```python
from build123d import *

# Parameters (mm, degrees)
SKETCH1_R           = 200
SKETCH1_R_2         = 20
BOSS_EXTRUDE1_DEPTH = 15
CUT_EXTRUDE1_DEPTH  = 30
FILLET1_R           = 50
SKETCH3_R           = 6.5
CUT_EXTRUDE2_DEPTH  = 50


with BuildPart() as part:
    # Sketch1 → Boss-Extrude1 (new body)
    with BuildSketch(Plane.XY):
        Circle(SKETCH1_R)
        with Locations((0, 156)):
            Circle(SKETCH1_R_2, mode=Mode.SUBTRACT)
        with Locations((135.09996299, -78)):
            Circle(SKETCH1_R_2, mode=Mode.SUBTRACT)
        with Locations((-135.09996299, -78)):
            Circle(SKETCH1_R_2, mode=Mode.SUBTRACT)
    extrude(amount=BOSS_EXTRUDE1_DEPTH)

    # Sketch2 → Cut-Extrude1 (cut)
    with BuildSketch(Plane.XY.offset(15)):
        with BuildLine():
            Line((-45.962666587, -116.432743419), (-177.651298468, -273.373143566))
            Line((-177.651298468, -273.373143566), (100.686015144, -181.64949066))
            Line((100.686015144, -181.64949066), (45.962666587, -116.432743419))
            ThreePointArc((45.962666587, -116.432743419), (0, -95), (-45.962666587, -116.432743419))
        make_face()
        with BuildLine():
            Line((-77.852380339, 98.0212086), (-147.922437807, 290.537109271))
            Line((-147.922437807, 290.537109271), (-207.656081069, 3.62809841))
            Line((-207.656081069, 3.62809841), (-123.815046927, 18.411534819))
            ThreePointArc((-123.815046927, 18.411534819), (-82.27241336, 47.5), (-77.852380339, 98.0212086))
        make_face()
        with BuildLine():
            Line((123.815046927, 18.411534819), (325.573736275, -17.163965705))
            Line((325.573736275, -17.163965705), (106.970065924, 178.021392251))
            Line((106.970065924, 178.021392251), (77.852380339, 98.0212086))
            ThreePointArc((77.852380339, 98.0212086), (82.27241336, 47.5), (123.815046927, 18.411534819))
        make_face()
    extrude(amount=-CUT_EXTRUDE1_DEPTH, mode=Mode.SUBTRACT)

    # Fillet1
    fillet1_edges = [part.edges().sort_by_distance(p)[0] for p in [
        (199.937763867, 4.989045978, 7.5),
        (104.289522491, 170.656659696, 7.5),
        (-104.289522491, 170.656659696, 7.5),
        (-199.937763867, 4.989045978, 7.5),
        (-95.648241376, -175.645705674, 7.5),
        (95.648241376, -175.645705674, 7.5),
    ]]
    fillet(fillet1_edges, radius=FILLET1_R)

    # Sketch3 → Cut-Extrude2 (cut)
    with BuildSketch(Plane.XY.offset(15)):
        with Locations((0, 30)):
            Circle(SKETCH3_R)
        with Locations((25.980762114, -15)):
            Circle(SKETCH3_R)
        with Locations((-25.980762114, -15)):
            Circle(SKETCH3_R)
    extrude(amount=-CUT_EXTRUDE2_DEPTH, mode=Mode.SUBTRACT)


solid = part.part
```
Read the model definition and answer for the solid it produces. Units are mm, in the model's axes. A direction names the side the tool comes from. Coordinates: 2 decimals unless noted, no trailing zeros. Write each loop counter-clockwise with the first axis right and the second up, starting at its lowest first coordinate (ties: lowest second). Pieces come first, ordered by that corner, then holes. Notation, with made-up numbers: (17, -14) - (64, -14) arc R12 ccw to (64, 9) - close; hole circle Ø10 at (-24.75, -38.75). An arc over 180 degrees is marked (long way). Answer as a JSON object with one key per item and string values. Group by question number.
1. A cutting plane is placed at C-C (y = -78). Determine the outline of the cut face in (x, z), plus the area to 3 significant figures.
2. A cutting plane is placed at B-B (z = 11.5). Determine the outline of the cut face in (x, y).
3. Which of the six approach directions +Z, -Z, +X, -X, +Y, -Y give full straight-line access (tool end or side, diameter ignored) to faces 1 (the flat face through (-55.756, -128.104, 7.605)), 2 (the flat face through (-83.063, 112.338, 7.605)), 3 (the flat face through (-3, -16, 0)), 4 (the cylindrical face through (0.8, 200, 7.4)), 5 (the flat face through (83.21, 112.74, 7.6))?
4. A cutting plane is placed at D-D (y = 156). Determine the outline of the cut face in (x, z), plus the area to 3 significant figures.
5. Each of these flat-tipped pins is pushed along its axis until it touches: P1, Ø8, axis at x = 25.98, y = -15, coming from the -Z side; P2, Ø5, axis at x = 133.5, z = 5, coming from the +Y side; P3, Ø4, axis at x = -33.5, z = 11.5, coming from the -Y side; P4, Ø2, axis at y = -39, z = 6.5, coming from the -X side. Where does it stop, or does it pass through?
6. The mould has two halves that part along X. Classify faces 6 (the flat face through (-139.2, 15.7, 7.6)), 7 (the flat face through (56.034, -128.436, 7.605)), 8 (the flat face through (138.819, 15.766, 7.605)): +X half, -X half, draft (parallel to the pull), parting line (faces both ways), or undercut.
7. Consider L1, parallel to Y at x = 0, z = 3.5; L2, parallel to Y at x = -5, z = 6.5; L3, parallel to Y at x = 123.5, z = 5.5. Determine where each line is inside the solid, lowest interval first. Write a range as [from, to].
8. A cutting plane is placed at A-A (x = 0). Determine the outline of the cut face in (y, z).
Worked out:
{
 "1": {"outline": "(-184.16, 0) - (-155.1, 0) - (-155.1, 15) - (-184.16, 15) - close; (-115.1, 0) - (115.1, 0) - (115.1, 15) - (-115.1, 15) - close; (155.1, 0) - (184.16, 0) - (184.16, 15) - (155.1, 15) - close", "area": "4,320 mm²"},
 "2": {"outline": "(-194.09, -48.26) arc R200 ccw to (-138.84, -143.96) arc R50 ccw to (-65.83, -140.11) - (-45.96, -116.43) arc R60 cw to (45.96, -116.43) - (65.83, -140.11) arc R50 ccw to (138.84, -143.96) arc R200 ccw to (194.09, -48.26) arc R50 ccw to (154.25, 13.05) - (123.82, 18.41) arc R60 cw to (77.85, 98.02) - (88.42, 127.06) arc R50 ccw to (55.25, 192.22) arc R200 ccw to (-55.25, 192.22) arc R50 ccw to (-88.42, 127.06) - (-77.85, 98.02) arc R60 cw to (-123.82, 18.41) - (-154.25, 13.05) arc R50 ccw to start; hole circle Ø40 at (-135.1, -78); hole circle Ø13 at (-25.98, -15); hole circle Ø40 at (0, 156); hole circle Ø13 at (0, 30); hole circle Ø13 at (25.98, -15); hole circle Ø40 at (135.1, -78)"},
 "3": {"face 1": "+Z, -Z, -Y", "face 2": "+Z, -Z, -X", "face 3": "-Z, +X, -X, +Y, -Y", "face 4": "+Z, -Z, +Y", "face 5": "+Z, -Z, +X"},
 "4": {"outline": "(-90.02, 0) - (-20, 0) - (-20, 15) - (-90.02, 15) - close; (20, 0) - (90.02, 0) - (90.02, 15) - (20, 15) - close", "area": "2,100 mm²"},
 "5": {"P1": "passes through", "P2": "stops at y = 17.14", "P3": "stops at y = -106.63", "P4": "stops at x = -195.53"},
 "6": {"face 6": "-X half", "face 7": "undercut", "face 8": "+X half"},
 "7": {"L1": "y = [-95, 23.5], [36.5, 136], [176, 200]", "L2": "y = [-95.21, 25.85], [34.15, 136.64], [175.36, 199.94]", "L3": "y = [-154.06, -94.29], [-61.71, 18.47]"},
 "8": {"outline": "(-95, 0) - (23.5, 0) - (23.5, 15) - (-95, 15) - close; (36.5, 0) - (136, 0) - (136, 15) - (36.5, 15) - close; (176, 0) - (200, 0) - (200, 15) - (176, 15) - close"}
}
